Work out the finished part from the listing and answer in its coordinate system (mm). Face numbers are marked on the shaded views. A direction names the side the tool comes from. Round coordinates to 2 decimals unless told otherwise and drop trailing zeros. Order: outer loops, then holes, each group sorted by start corner. A loop starts at its lowest first (then second) coordinate and runs counter-clockwise, first axis right, second up. Notation, with made-up numbers: M 34.5,32 L 86.5,32 A29 ccw 86.5,59 Z; hole C 41.25,-8 d6. An arc over 180 degrees is marked long. Return JSON: item names as keys, results as strings.
from build123d import *

# Parameters (mm, degrees)
EXTRUDE_1_DEPTH     = 20
SKETCH_2_R          = 3
CUT_EXTRUDE_1_DEPTH = 209.386659842


with BuildPart() as part:
    # 草图1 → 拉伸-薄壁1 (new body)
    with BuildSketch(Plane.XY):
        with BuildLine():
            Line((0, 0), (27.5, 0))
            ThreePointArc((27.5, 0), (32.803300859, 2.196699141), (35, 7.5))
            Line((35, 7.5), (35, 42.5))
            ThreePointArc((35, 42.5), (37.196699141, 47.803300859), (42.5, 50))
            Line((42.5, 50), (157.5, 50))
            ThreePointArc((157.5, 50), (162.803300859, 47.803300859), (165, 42.5))
            Line((165, 42.5), (165, 7.5))
            ThreePointArc((165, 7.5), (167.196699141, 2.196699141), (172.5, 0))
            Line((172.5, 0), (200, 0))
            Line((200, 0), (200, -5))
            Line((200, -5), (172.5, -5))
            ThreePointArc((172.5, -5), (163.661165235, -1.338834765), (160, 7.5))
            Line((160, 7.5), (160, 42.5))
            ThreePointArc((160, 42.5), (159.267766953, 44.267766953), (157.5, 45))
            Line((157.5, 45), (42.5, 45))
            ThreePointArc((42.5, 45), (40.732233047, 44.267766953), (40, 42.5))
            Line((40, 42.5), (40, 7.5))
            ThreePointArc((40, 7.5), (36.338834765, -1.338834765), (27.5, -5))
            Line((27.5, -5), (0, -5))
            Line((0, -5), (0, 0))
        make_face()
    extrude(amount=EXTRUDE_1_DEPTH)

    # 草图2 → 切除-拉伸1 (cut, through all)
    with BuildSketch(Plane.XZ.offset(5)):
        with Locations(Location((15, 10, 0), (0, 0, 270))):
            Circle(SKETCH_2_R)
        with Locations(Location((185, 10, 0), (0, 0, 270))):
            Circle(SKETCH_2_R)
    extrude(amount=-CUT_EXTRUDE_1_DEPTH, mode=Mode.SUBTRACT)


solid = part.part
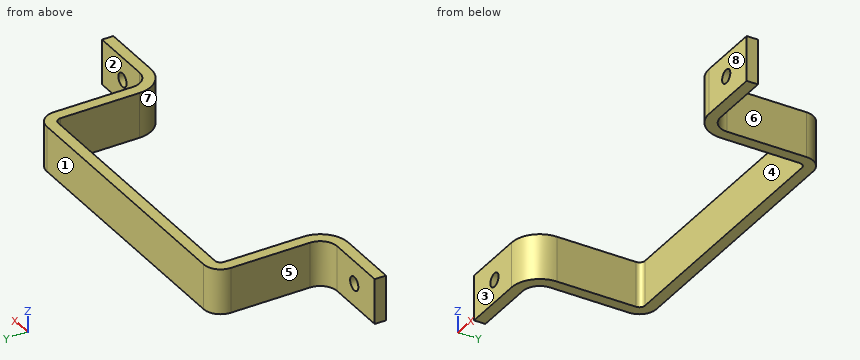
Item 1: The mould has two halves that part along X. Classify the marked faces 6, 7 and 8: pulls with the +X half, pulls with the -X half, needs draft (parallel to the pull), parting line crosses it, or undercut.
Output:
{"face 6": "pulls with the +X half", "face 7": "undercut", "face 8": "needs draft"}
Item 2: Each of these flat-tipped pins is pushed along its axis until it touches: pin 1 (10 mm diameter, centred on x = 13.5, z = 9.5, fed in from +Y); pin 2 (6 mm diameter, centred on y = 26.5, z = 11, fed in from -X); pin 3 (6 mm diameter, centred on x = 106.5, z = 18, fed in from -Y); pin 4 (5 mm diameter, centred on x = 15, z = 10, fed in from +Y). Where does it stop, or does it pass through?
Output:
{"pin 1": "stops at y = 0", "pin 2": "stops at x = 35", "pin 3": "stops at y = 45", "pin 4": "passes through"}
Item 3: Find section B-B (z = 10). Determine the outline of the cut face in (x, y).
Output:
{"outline": "M 0,-5 L 12,-5 L 12,0 L 0,0 Z; M 18,-5 L 27.5,-5 A12.5 ccw 40,7.5 L 40,42.5 A2.5 cw 42.5,45 L 157.5,45 A2.5 cw 160,42.5 L 160,7.5 A12.5 ccw 172.5,-5 L 182,-5 L 182,0 L 172.5,0 A7.5 cw 165,7.5 L 165,42.5 A7.5 ccw 157.5,50 L 42.5,50 A7.5 ccw 35,42.5 L 35,7.5 A7.5 cw 27.5,0 L 18,0 Z; M 188,-5 L 200,-5 L 200,0 L 188,0 Z"}
Item 4: Which of the six approach directions +Z, -Z, +X, -X, +Y, -Y give full straight-line access (tool end or side, diameter ignored) to the marked faces 1, 2, 3, 4 and 5?
Output:
{"face 1": "+Z, -Z, +X, -X, +Y", "face 2": "+Z, -Z, +X, +Y", "face 3": "+Z, -Z, +X, -X, -Y", "face 4": "+Z, -Z, -Y", "face 5": "+Z, -Z, -X, +Y"}
Item 5: Find section A-A (x = 15). Determine the outline of the cut face in (y, z).
Output:
{"outline": "M -5,0 L 0,0 L 0,7 L -5,7 Z; M -5,13 L 0,13 L 0,20 L -5,20 Z"}
Item 6: Consider line 1 along X through (y, z) = (40, 4.25); line 2 along X through (y, z) = (-1.25, 10); line 3 along X through (y, z) = (-3.15, 10). Determine where each line is inside the solid, lowest interval first. Write a range as [from, to].
Output:
{"line 1": "x = [35, 40], [160, 165]", "line 2": "x = [0, 12], [18, 36.43], [163.57, 182], [188, 200]", "line 3": "x = [0, 12], [18, 34.04], [165.96, 182], [188, 200]"}
Item 7: Find section D-D (x = 132.5). Determine the outline of the cut face in (y, z), plus the area to 3 significant figures.
Output:
{"outline": "M 45,0 L 50,0 L 50,20 L 45,20 Z", "area": "100 mm^2"}
Item 8: Find section C-C (y = 32.5). Determine the outline of the cut face in (x, z).
Output:
{"outline": "M 35,0 L 40,0 L 40,20 L 35,20 Z; M 160,0 L 165,0 L 165,20 L 160,20 Z"}
